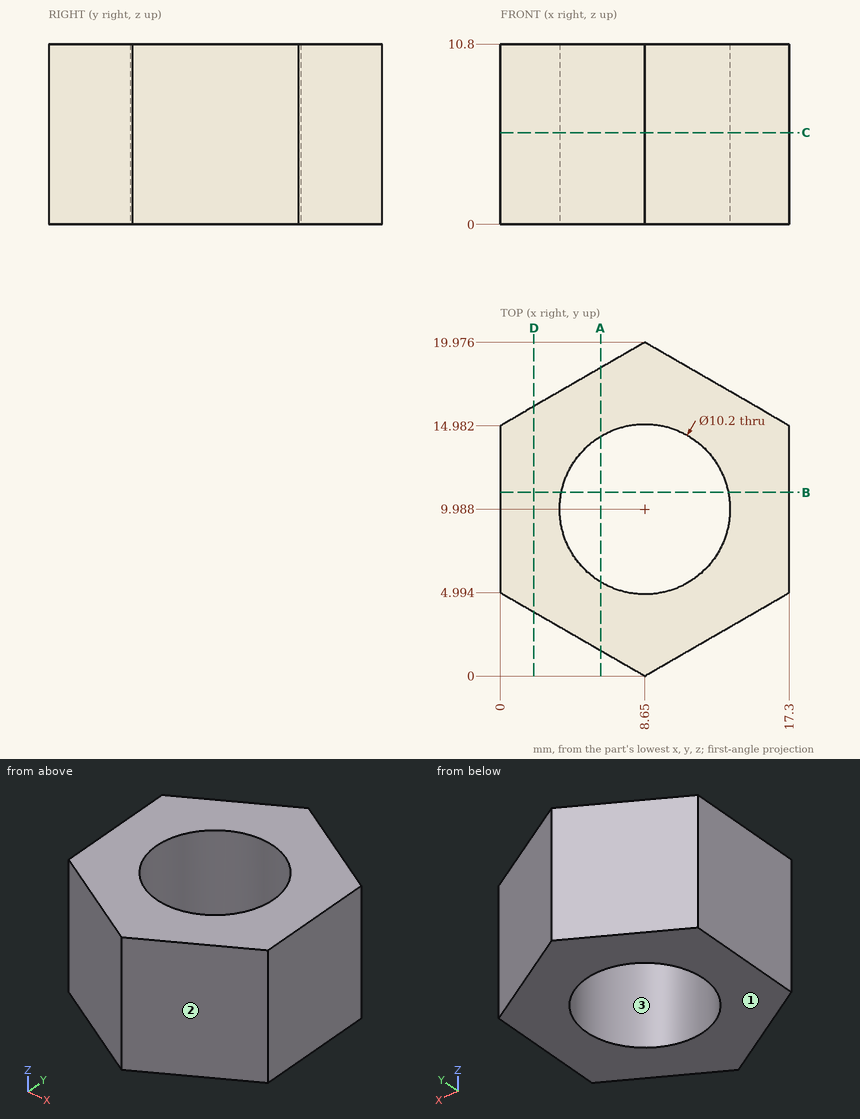
Verification items for this drawing (mm, ordinates from the low corner). Coordinates: 2 decimals unless noted, no trailing zeros. Loops run counter-clockwise (first coordinate to the right, second up) from the corner with the lowest first, then second, coordinate; pieces in that order, holes last. Notation, with made-up numbers: (46, -12.5) - (53, -12.5) arc R18 ccw to (53, 21.5) - close; hole circle Ø5 at (33, 56). An arc over 180 degrees is marked (long way). Answer as a JSON object with one key per item and string values.
(1) Cross-section at D-D, the plane x = 2. Record the boundary of the cut face in (y, z), then the cut area to 3 significant figures.
Response:
{"outline": "(3.84, 0) - (16.14, 0) - (16.14, 10.8) - (3.84, 10.8) - close", "area": "133 mm²"}
(2) Cross-section at A-A, the plane x = 6. Record the boundary of the cut face in (y, z) (1 decimal).
Response:
{"outline": "(1.5, 0) - (5.6, 0) - (5.6, 10.8) - (1.5, 10.8) - close; (14.3, 0) - (18.4, 0) - (18.4, 10.8) - (14.3, 10.8) - close"}
(3) Cross-section at C-C, the plane z = 5.5. Record the boundary of the cut face in (x, y).
Response:
{"outline": "(0, 4.99) - (8.65, 0) - (17.3, 4.99) - (17.3, 14.98) - (8.65, 19.98) - (0, 14.98) - close; hole circle Ø10.2 at (8.65, 9.99)"}
(4) Go/stop test with flat-tipped pins: pin 1 Ø4 at (x, z) = (8, 7) entering from -Y; pin 2 Ø1 at (x, z) = (6, 1.5) entering from -Y. Record where each tip stops, or that it passes through.
Response:
{"pin 1": "stops at y = 0", "pin 2": "stops at y = 1.24"}
(5) Cross-section at B-B, the plane y = 11. Record the boundary of the cut face in (x, z).
Response:
{"outline": "(0, 0) - (3.65, 0) - (3.65, 10.8) - (0, 10.8) - close; (13.65, 0) - (17.3, 0) - (17.3, 10.8) - (13.65, 10.8) - close"}
(6) Scan lines: line 1 along X through (y, z) = (9.75, 9.5) (1 decimal); line 2 along Y through (x, z) = (12, 4.25) (1 decimal); line 3 along X through (y, z) = (6.5, 1.25). Record each from-to range of solid material in increasing order.
Response:
{"line 1": "x = 0 to 3.6, 13.7 to 17.3", "line 2": "y = 1.9 to 6.1, 13.8 to 18", "line 3": "x = 0 to 4.93, 12.37 to 17.3"}
(7) Mould release check, pull along Y, two halves, no side actions. Record for the marked faces 1, 2 and 3: pulls with the +Y half, pulls with the -Y half, needs draft (parallel to the pull), parting line crosses it, or undercut.
Response:
{"face 1": "needs draft", "face 2": "pulls with the -Y half", "face 3": "undercut"}
